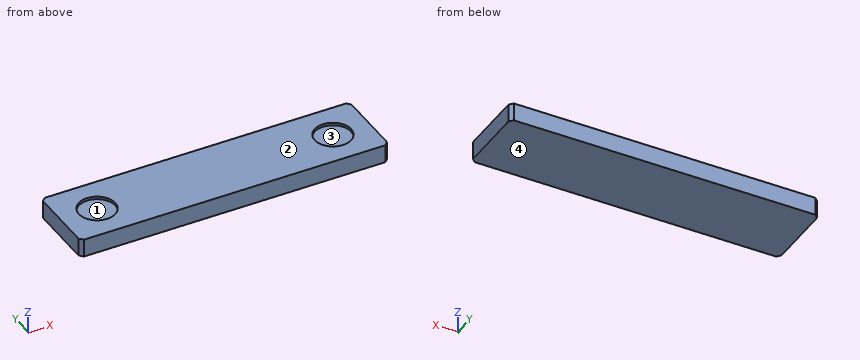
from build123d import *

# Parameters (mm, degrees)
SKETCH_1_W          = 170
SKETCH_1_H          = 40
EXTRUDE_1_DEPTH     = 10
SKETCH_2_R          = 10
CUT_EXTRUDE_1_DEPTH = 1.5
CHAMFER_1_SIZE      = 2


with BuildPart() as part:
    # 草图1 → 凸台-拉伸1 (new body)
    with BuildSketch(Plane.XY):
        Rectangle(SKETCH_1_W, SKETCH_1_H)
    extrude(amount=EXTRUDE_1_DEPTH)

    # 草图2 → 切除-拉伸1 (cut)
    with BuildSketch(Plane.XY.offset(10)):
        with Locations((-65, 0)):
            Circle(SKETCH_2_R)
        with Locations((65, 0)):
            Circle(SKETCH_2_R)
    extrude(amount=-CUT_EXTRUDE_1_DEPTH, mode=Mode.SUBTRACT)

    # 倒角1
    chamfer_1_edges = [part.edges().sort_by_distance(p)[0] for p in [
        (85, -20, 5),
        (-85, -20, 5),
        (-85, 20, 5),
        (85, 20, 5),
    ]]
    chamfer(chamfer_1_edges, length=CHAMFER_1_SIZE)


solid = part.part
Geometry check sheet. Reference: the model listing, model coordinates, mm. Face numbers are marked on the shaded views. A direction names the side the tool comes from. Round coordinates to 2 decimals unless told otherwise and drop trailing zeros. Order: outer loops, then holes, each group sorted by start corner. A loop starts at its lowest first (then second) coordinate and runs counter-clockwise, first axis right, second up. Notation, with made-up numbers: M -2,0 L 31,0 A22 ccw 31,28 Z; hole C -3.5,26.5 d7. An arc over 180 degrees is marked long. Write each question's results on one line, items separated by ' | '. Start each with the question number.
1. Set-up check for the marked faces 1 and 2: record each of +Z, -Z, +X, -X, +Y, -Y from which the full face is reachable in a straight line by a thin tool's end or side.
2. Cross-section at A-A on y = 0. Record the boundary of the cut face in (x, z).
3. Material ranges on L1, parallel to Y at x = -65, z = 9.2; L2, parallel to Z at x = 70, y = 7, recorded low to high. Write a range as from..to.
4. Cross-section at B-B on x = -65. Record the boundary of the cut face in (y, z).
5. Go/stop test with flat-tipped pins: P1, Ø10, axis at x = -69, y = -2.5, coming from the +Z side; P2, Ø23, axis at x = 65, y = 0, coming from the +Z side. Record where each tip stops, or that it passes through.
6. Draft check along X on the marked faces 3 and 4. Enter one of: pulls with the +X half, pulls with the -X half, needs draft (parallel to the pull), parting line crosses it, or undercut.
7. Cross-section at C-C on x = 68. Record the boundary of the cut face in (y, z), plus the area to 3 significant figures.
Resolved:
1) face 1: +Z | face 2: +Z, +X, -X, +Y, -Y
2) outline: M -85,0 L 85,0 L 85,10 L 75,10 L 75,8.5 L 55,8.5 L 55,10 L -55,10 L -55,8.5 L -75,8.5 L -75,10 L -85,10 Z
3) L1: -20..-10, 10..20 | L2: 0..8.5
4) outline: M -20,0 L 20,0 L 20,10 L 10,10 L 10,8.5 L -10,8.5 L -10,10 L -20,10 Z
5) P1: z = 8.5 | P2: z = 10
6) face 3: undercut | face 4: needs draft
7) outline: M -20,0 L 20,0 L 20,10 L 9.54,10 L 9.54,8.5 L -9.54,8.5 L -9.54,10 L -20,10 Z | area: 371 mm2
